from build123d import *

# Parameters (mm, degrees)
SKETCH1_W                = 450
SKETCH1_H                = 280
BOSS_EXTRUDE1_DEPTH      = 180
BOSS_EXTRUDE2_DEPTH      = 40
BOSS_EXTRUDE2_DEPTH_BACK = 220
SKETCH2_W                = 550
SKETCH2_H                = 30


with BuildPart() as part:
    # Sketch1 → Boss-Extrude1 (new body)
    with BuildSketch(Plane(origin=(0, 0, 0), x_dir=(1, 0, 0), z_dir=(0, 1, 0))):
        with Locations((225, -140)):
            Rectangle(SKETCH1_W, SKETCH1_H)
    extrude(amount=BOSS_EXTRUDE1_DEPTH)

    # Sketch2 → Boss-Extrude2 (add, two sides: drawn at the far end of the back side and taken through both)
    with BuildSketch(Plane.XZ.offset(-BOSS_EXTRUDE2_DEPTH_BACK)):
        with Locations((225, 15)):
            Rectangle(SKETCH2_W, SKETCH2_H)
    extrude(amount=BOSS_EXTRUDE2_DEPTH + BOSS_EXTRUDE2_DEPTH_BACK)


solid = part.part
Verification items for the finished model (mm, model axes). A direction names the side the tool comes from. Round coordinates to 2 decimals unless told otherwise and drop trailing zeros. Loops run counter-clockwise (first coordinate to the right, second up) from the corner with the lowest first, then second, coordinate; pieces in that order, holes last. Notation, with made-up numbers: (46.25, 48) - (99.25, 48) arc R32 cw to (99.25, 78) - close; hole circle Ø7 at (-9.5, 88.5). An arc over 180 degrees is marked (long way). Write item = value, one per line.
Q1. Sectioned sample at D-D on y = -23.5. Record the boundary of the cut face in (x, z).
Here are the results:
outline = (-50, 0) - (500, 0) - (500, 30) - (-50, 30) - close
Q2. Mould release check, pull along X, two halves, no side actions. Record for faces 5 (the flat face through (500, 92, 15)), 6 (the flat face through (-50, 92, 15)), 7 (the flat face through (221, -24, 30)): +X half, -X half, draft (parallel to the pull), parting line (faces both ways), or undercut.
Here are the results:
face_5 = +X half
face_6 = -X half
face_7 = draft
Q3. Tool access check on faces 1 (the flat face through (450, 89, 157)), 2 (the flat face through (222, 180, 153)), 3 (the flat face through (222, 0, 153)), 4 (the flat face through (0, 89, 157)). Record the directions out of +Z, -Z, +X, -X, +Y, -Y that give a thin tool (end or side, any length) a straight path to the whole face; none if there is none.
Here are the results:
face_1 = +Z, +X, +Y, -Y
face_2 = +Z, +X, -X, +Y
face_3 = +Z, +X, -X, -Y
face_4 = +Z, -X, +Y, -Y
Q4. Sectioned sample at A-A on x = 270.5. Record the boundary of the cut face in (y, z), plus the area to 3 significant figures.
Here are the results:
outline = (-40, 0) - (220, 0) - (220, 30) - (180, 30) - (180, 280) - (0, 280) - (0, 30) - (-40, 30) - close
area = 52,800 mm^2
Q5. Material ranges on L1, parallel to X at y = 127.5, z = 145.5; L2, parallel to Y at x = 304, z = 134; L3, parallel to Z at x = 454, y = 167, recorded low to high.
Here are the results:
L1 = 0 to 450
L2 = 0 to 180
L3 = 0 to 30
Q6. Sectioned sample at C-C on z = 204.5. Record the boundary of the cut face in (x, y).
Here are the results:
outline = (0, 0) - (450, 0) - (450, 180) - (0, 180) - close
Q7. Depth check by flat-ended pin: pin 1 (1 mm diameter, centred on x = 13, z = 123, fed in from +Y); pin 2 (6 mm diameter, centred on x = 266.5, z = 161, fed in from -Y); pin 3 (12 mm diameter, centred on y = 145, z = 169.5, fed in from +X); pin 4 (12 mm diameter, centred on x = 144.5, y = 71.5, fed in from -Z). Enter the tip coordinate at first touch or a pass-through.
Here are the results:
pin_1 = 180
pin_2 = 0
pin_3 = 450
pin_4 = 0
Q8. Sectioned sample at B-B on y = 96. Record the boundary of the cut face in (x, z), plus the area to 3 significant figures.
Here are the results:
outline = (-50, 0) - (500, 0) - (500, 30) - (450, 30) - (450, 280) - (0, 280) - (0, 30) - (-50, 30) - close
area = 129,000 mm^2
